Work out the finished part from the listing and answer in its coordinate system (mm). Face numbers are marked on the shaded views. Give positions to 0.01 mm unless a question says otherwise; leave off trailing zeros. Loops run counter-clockwise (first coordinate to the right, second up) from the corner with the lowest first, then second, coordinate; pieces in that order, holes last. Notation, with made-up numbers: M -9.75,-33 L 37.25,-33 A7 ccw 37.25,-27 Z; hole C -24.5,-15 d5. An arc over 180 degrees is marked long. Write item = value, one per line. Start each with the question number.
1. Consider L1, parallel to Z at x = 5.25, y = 4.25; L2, parallel to Y at x = 0, z = 6.1. Determine where each line is inside the solid, lowest interval first. Write a range as [from, to].
2. The mould has two halves that part along Y. Classify the marked faces 1, 2 and 3: released by +Y, released by -Y, zero draft, split by the parting line, or undercut.
3. Section A-A on y = 0 is taken. Determine the outline of the cut face in (x, z), plus the area to 3 significant figures.
4. Section D-D on x = -8.5 is taken. Determine the outline of the cut face in (y, z).
5. Section C-C on z = 0 is taken. Determine the outline of the cut face in (x, y).
6. Flat-ended cylindrical pins translate along their axes: pin 1 Ø9.5 at (x, y) = (0, 0) entering from +Z; pin 2 Ø1.5 at (x, z) = (9, -2) entering from -Y. Find the tip coordinate at first contact, or state that the pin passes through.
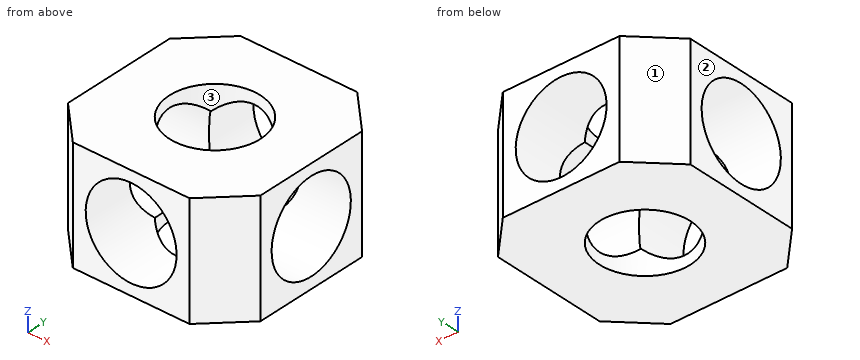
```python
from build123d import *

# Parameters (mm, degrees)
NUT_BODY_PROFILE_W     = 25.4
NUT_BODY_PROFILE_H     = 25.4
NUT_BODY_DEPTH         = 7.5
EDGE_CHAMFERS_5MM_SIZE = 5
AXIAL_BORE_PROFILE_R   = 6
AXIAL_BORE_12_DEPTH    = 15
CROSS_BORE_A_PROFILE_R = 6
CROSS_BORE_A_12_DEPTH  = 30.37175514
CROSS_BORE_B_PROFILE_R = 6
CROSS_BORE_B_12_DEPTH  = 30.37175514


with BuildPart() as part:
    # Nut Body Profile → Nut Body (new, symmetric)
    with BuildSketch(Plane.XY):
        Rectangle(NUT_BODY_PROFILE_W, NUT_BODY_PROFILE_H)
    extrude(amount=NUT_BODY_DEPTH, both=True)

    # Edge Chamfers 5mm
    edge_chamfers_5mm_edges = [part.edges().sort_by_distance(p)[0] for p in [
        (12.7, -12.7, 0),
        (-12.7, -12.7, 0),
        (-12.7, 12.7, 0),
        (12.7, 12.7, 0),
    ]]
    chamfer(edge_chamfers_5mm_edges, length=EDGE_CHAMFERS_5MM_SIZE)

    # Axial Bore Profile → Axial Bore Ø12 (cut)
    with BuildSketch(Plane(origin=(0, 0, -7.5), x_dir=(-1, 0, 0), z_dir=(0, 0, -1))):
        Circle(AXIAL_BORE_PROFILE_R)
    extrude(amount=-AXIAL_BORE_12_DEPTH, mode=Mode.SUBTRACT)

    # Cross Bore A Profile → Cross Bore A Ø12 (cut, through all)
    with BuildSketch(Plane.ZY.offset(12.7)):
        Circle(CROSS_BORE_A_PROFILE_R)
    extrude(amount=-CROSS_BORE_A_12_DEPTH, mode=Mode.SUBTRACT)

    # Cross Bore B Profile → Cross Bore B Ø12 (cut, through all)
    with BuildSketch(Plane(origin=(0, 12.7, 0), x_dir=(1, 0, 0), z_dir=(0, 1, 0))):
        with Locations(Location((0, 0, 0), (0, 0, 270))):
            Circle(CROSS_BORE_B_PROFILE_R)
    extrude(amount=-CROSS_BORE_B_12_DEPTH, mode=Mode.SUBTRACT)


solid = part.part
```
Verdict:
q1.L1 = [-7.5, -4.24], [4.24, 7.5]
q1.L2 = [-12.7, -6], [6, 12.7]
q2.face_1 = released by +Y
q2.face_2 = zero draft
q2.face_3 = undercut
q3.outline = M -12.7,-7.5 L -6,-7.5 L -6,-6 L -12.7,-6 Z; M -12.7,6 L -6,6 L -6,7.5 L -12.7,7.5 Z; M 6,-7.5 L 12.7,-7.5 L 12.7,-6 L 6,-6 Z; M 6,6 L 12.7,6 L 12.7,7.5 L 6,7.5 Z
q3.area = 40.2 mm2
q4.outline = M -11.9,-7.5 L 11.9,-7.5 L 11.9,7.5 L -11.9,7.5 Z; hole C 0,0 d12
q5.outline = M -12.7,-7.7 L -7.7,-12.7 L -6,-12.7 L -6,-6 L -12.7,-6 Z; M -12.7,6 L -6,6 L -6,12.7 L -7.7,12.7 L -12.7,7.7 Z; M 6,-12.7 L 7.7,-12.7 L 12.7,-7.7 L 12.7,-6 L 6,-6 Z; M 6,6 L 12.7,6 L 12.7,7.7 L 7.7,12.7 L 6,12.7 Z
q6.pin_1 = through
q6.pin_2 = -12.15
